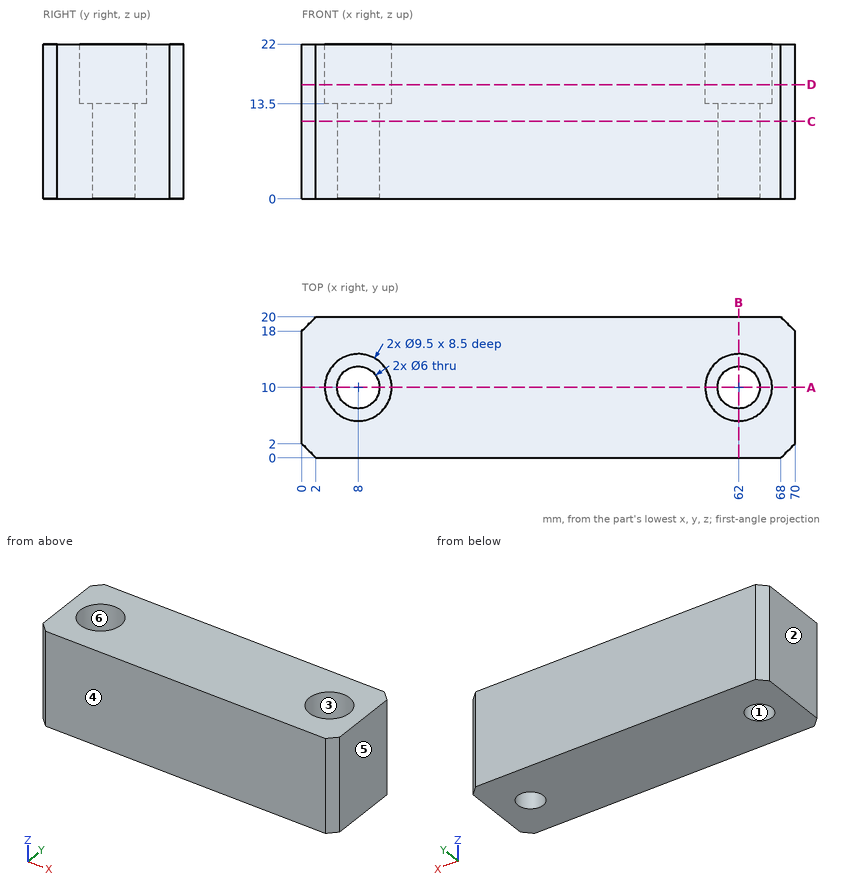
Verification items for this drawing (mm, ordinates from the low corner). A direction names the side the tool comes from. Coordinates: 2 decimals unless noted, no trailing zeros. Order: outer loops, then holes, each group sorted by start corner. A loop starts at its lowest first (then second) coordinate and runs counter-clockwise, first axis right, second up. Notation, with made-up numbers: M 79.5,26 L 122.5,26 A20 cw 122.5,52 Z; hole C 17.25,36 d3. An arc over 180 degrees is marked long. Answer as a JSON object with one key per item and string values.
Q1. Cross-section at C-C on z = 11. Record the cut outline in (x, y), and give its area (3 significant figures).
Results are:
{"outline": "M 0,2 L 2,0 L 68,0 L 70,2 L 70,18 L 68,20 L 2,20 L 0,18 Z; hole C 8,10 d6; hole C 62,10 d6", "area": "1,340 mm²"}
Q2. Scan lines: line 1 (X direction, y = 8.25, z = 17.25); line 2 (Y direction, x = 8, z = 3.25); line 3 (X direction, y = 8.25, z = 7.5). Record each from-to range of solid material in increasing order.
Results are:
{"line 1": "x = 0 to 3.58, 12.42 to 57.58, 66.42 to 70", "line 2": "y = 0 to 7, 13 to 20", "line 3": "x = 0 to 5.56, 10.44 to 59.56, 64.44 to 70"}
Q3. Cross-section at B-B on x = 62. Record the cut outline in (y, z), and give its area (3 significant figures).
Results are:
{"outline": "M 0,0 L 7,0 L 7,13.5 L 5.25,13.5 L 5.25,22 L 0,22 Z; M 13,0 L 20,0 L 20,22 L 14.75,22 L 14.75,13.5 L 13,13.5 Z", "area": "278 mm²"}
Q4. Depth check by flat-ended pin: pin 1 Ø5.5 at (x, y) = (8, 10) entering from +Z; pin 2 Ø7.5 at (x, y) = (62, 10) entering from +Z. Enter the tip coordinate at first touch or a pass-through.
Results are:
{"pin 1": "passes through", "pin 2": "stops at z = 13.5"}
Q5. Cross-section at D-D on z = 16.25. Record the cut outline in (x, y).
Results are:
{"outline": "M 0,2 L 2,0 L 68,0 L 70,2 L 70,18 L 68,20 L 2,20 L 0,18 Z; hole C 8,10 d9.5; hole C 62,10 d9.5"}
Q6. Tool access check on the marked faces 5 and 6. Record the directions out of +Z, -Z, +X, -X, +Y, -Y that give a thin tool (end or side, any length) a straight path to the whole face; none if there is none.
Results are:
{"face 5": "+Z, -Z, +X, +Y, -Y", "face 6": "+Z"}
Q7. Release check for a two-part mould opening along Y. For the marked faces 1, 2, 3 and 4 record: released by +Y, released by -Y, zero draft, split by the parting line, or undercut.
Results are:
{"face 1": "undercut", "face 2": "zero draft", "face 3": "undercut", "face 4": "released by -Y"}
Q8. Cross-section at A-A on y = 10. Record the cut outline in (x, z).
Results are:
{"outline": "M 0,0 L 5,0 L 5,13.5 L 3.25,13.5 L 3.25,22 L 0,22 Z; M 11,0 L 59,0 L 59,13.5 L 57.25,13.5 L 57.25,22 L 12.75,22 L 12.75,13.5 L 11,13.5 Z; M 65,0 L 70,0 L 70,22 L 66.75,22 L 66.75,13.5 L 65,13.5 Z"}
